```python
from build123d import *

# Parameters (mm, degrees)
SKETCH_1_W             = 58
SKETCH_1_H             = 95
EXTRUDE_1_DEPTH        = 5
CUT_EXTRUDE_1_DEPTH    = 10
HOLE_WIZARD_M5_1_D     = 4.2
HOLE_WIZARD_M5_1_DEPTH = 12.4
HOLE_WIZARD_M5_1_TIP   = 1.2618073
HOLE_WIZARD_M5_2_D     = 4.2
HOLE_WIZARD_M5_2_DEPTH = 12.4
HOLE_WIZARD_M5_2_TIP   = 1.2618073


with BuildPart() as part:
    # 草图1 → 凸台-拉伸1 (new, symmetric)
    with BuildSketch(Plane(origin=(0, 0, 0), x_dir=(1, 0, 0), z_dir=(0, 1, 0))):
        Rectangle(SKETCH_1_W, SKETCH_1_H)
    extrude(amount=EXTRUDE_1_DEPTH, both=True)

    # 草图2 → 切除-拉伸1 (cut)
    with BuildSketch(Plane(origin=(0, 5, 0), x_dir=(1, 0, 0), z_dir=(0, 1, 0))):
        Polygon((19, -47.5), (-29, 37.5), (-29, -47.5), align=None)
    extrude(amount=-CUT_EXTRUDE_1_DEPTH, mode=Mode.SUBTRACT)

    # M5 螺纹孔1
    with Locations(Plane(origin=(29, 0, 0), x_dir=(0, 0, -1), z_dir=(1, 0, 0))):
        with Locations((-37.5, 0), (22.5, 0)):
            Hole(HOLE_WIZARD_M5_1_D / 2, depth=HOLE_WIZARD_M5_1_DEPTH)
            with Locations((0, 0, -(HOLE_WIZARD_M5_1_DEPTH + HOLE_WIZARD_M5_1_TIP / 2))):  # 118° drill point
                Cone(0, HOLE_WIZARD_M5_1_D / 2, HOLE_WIZARD_M5_1_TIP, mode=Mode.SUBTRACT)

    # M5 螺纹孔2
    with Locations(Plane(origin=(0, 0, -47.5), x_dir=(-1, 0, 0), z_dir=(0, 0, -1))):
        with Locations((19, 0), (-21, 0)):
            Hole(HOLE_WIZARD_M5_2_D / 2, depth=HOLE_WIZARD_M5_2_DEPTH)
            with Locations((0, 0, -(HOLE_WIZARD_M5_2_DEPTH + HOLE_WIZARD_M5_2_TIP / 2))):  # 118° drill point
                Cone(0, HOLE_WIZARD_M5_2_D / 2, HOLE_WIZARD_M5_2_TIP, mode=Mode.SUBTRACT)


solid = part.part
```
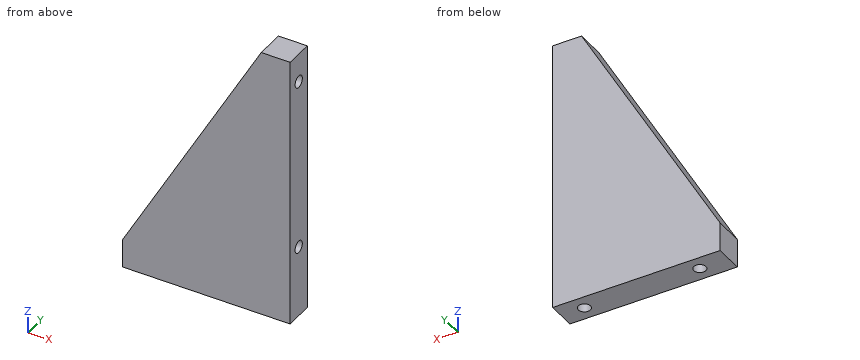
Verification items for the finished model (mm, model axes). Give positions to 0.01 mm unless a question says otherwise; leave off trailing zeros. Order: outer loops, then holes, each group sorted by start corner. A loop starts at its lowest first (then second) coordinate and runs counter-clockwise, first axis right, second up. Notation, with made-up numbers: M 21,38.5 L 44,38.5 A28 ccw 44,75.5 Z; hole C 27.25,9 d11. An arc over 180 degrees is marked long. Answer in a Markdown table with one row per item. Add a question column.
Item 1: Scan lines: probe 1 along Z at (x, y) = (26.25, 0); probe 2 along X at (y, z) = (0, -44.5); probe 3 along Z at (x, y) = (22.5, 0). Record each from-to range of solid material in increasing order. Write a range as from..to.
Item 2: Section check A-A, the plane y = -3.5. Enter the section's corners in (x, z).
Item 3: Section check B-B, the plane x = -7. Enter the section's corners in (y, z).
Item 4: Gauge pin test, flat ends, axial feed: pin 1 (1.5 mm diameter, centred on x = -17.5, y = -3, fed in from +Z); pin 2 (3.5 mm diameter, centred on y = 0, z = 37.5, fed in from -X); pin 3 (3.5 mm diameter, centred on x = -19, y = 0, fed in from +Z). Record the tip position at first contact, or that the pin passes through.
Item 5: Section check C-C, the plane z = 21. Enter the section's corners in (x, y).
Filled sheet:
| question | item | result |
|---|---|---|
| 1 | probe 1 | z = -47.5..-24.6, -20.4..35.4, 39.6..47.5 |
| 1 | probe 2 | x = -29..-21.1, -16.9..18.9, 23.1..29 |
| 1 | probe 3 | z = -34.74..-24.6, -20.4..35.4, 39.6..47.5 |
| 2 | outline | M -29,-47.5 L 29,-47.5 L 29,47.5 L 19,47.5 L -29,-37.5 Z |
| 3 | outline | M -5,-47.5 L 5,-47.5 L 5,1.46 L -5,1.46 Z |
| 4 | pin 1 | stops at z = -15.81 |
| 4 | pin 2 | stops at x = 12.36 |
| 4 | pin 3 | stops at z = -16.69 |
| 5 | outline | M 4.04,-5 L 29,-5 L 29,5 L 4.04,5 Z |
